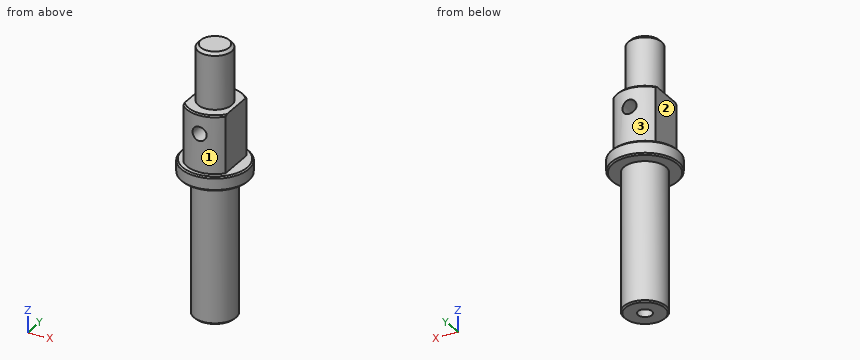
```python
from build123d import *

# Parameters (mm, degrees)
SKETCH_1_R             = 7.5
EXTRUDE_1_DEPTH        = 49.5
SKETCH_2_R             = 12
EXTRUDE_2_DEPTH        = 5
SKETCH_3_R             = 10
EXTRUDE_3_DEPTH        = 20.5
SKETCH_4_R             = 6
EXTRUDE_4_DEPTH        = 20
HOLE_WIZARD_M6_1_D     = 5
HOLE_WIZARD_M6_1_DEPTH = 15
HOLE_WIZARD_M6_1_TIP   = 1.502151548
CHAMFER_1_SIZE         = 0.5
CHAMFER_2_SIZE         = 1
CHAMFER_3_SIZE         = 0.5
SKETCH_7_W             = 26.460285879
SKETCH_7_H             = 26.47281766
SKETCH_7_W_2           = 19.498728734
SKETCH_7_H_2           = 28.747669346
CUT_EXTRUDE_1_DEPTH    = 52
HOLE_WIZARD_M6_2_D     = 5


with BuildPart() as part:
    # 草图1 → 凸台-拉伸1 (new body)
    with BuildSketch(Plane.XY):
        Circle(SKETCH_1_R)
    extrude(amount=EXTRUDE_1_DEPTH)

    # 草图2 → 凸台-拉伸2 (add)
    with BuildSketch(Plane.XY.offset(49.5)):
        Circle(SKETCH_2_R)
    extrude(amount=EXTRUDE_2_DEPTH)

    # 草图3 → 凸台-拉伸3 (add)
    with BuildSketch(Plane.XY.offset(54.5)):
        Circle(SKETCH_3_R)
    extrude(amount=EXTRUDE_3_DEPTH)

    # 草图4 → 凸台-拉伸4 (add)
    with BuildSketch(Plane.XY.offset(75)):
        Circle(SKETCH_4_R)
    extrude(amount=EXTRUDE_4_DEPTH)

    # M6 螺纹孔1
    with Locations(Plane(origin=(0, 0, 0), x_dir=(-1, 0, 0), z_dir=(0, 0, -1))):
        with Locations((0, 0)):
            Hole(HOLE_WIZARD_M6_1_D / 2, depth=HOLE_WIZARD_M6_1_DEPTH)
            with Locations((0, 0, -(HOLE_WIZARD_M6_1_DEPTH + HOLE_WIZARD_M6_1_TIP / 2))):  # 118° drill point
                Cone(0, HOLE_WIZARD_M6_1_D / 2, HOLE_WIZARD_M6_1_TIP, mode=Mode.SUBTRACT)

    # 倒角1
    chamfer_1_edges = [part.edges().sort_by_distance(p)[0] for p in [
        (-7.5, 0, 0),
        (-12, 0, 49.5),
        (-12, 0, 54.5),
    ]]
    chamfer(chamfer_1_edges, length=CHAMFER_1_SIZE)

    # 倒角2
    chamfer_2_edges = [part.edges().sort_by_distance(p)[0] for p in [
        (-6, 0, 95),
    ]]
    chamfer(chamfer_2_edges, length=CHAMFER_2_SIZE)

    # 倒角3
    chamfer_3_edges = [part.edges().sort_by_distance(p)[0] for p in [
        (-10, 0, 75),
    ]]
    chamfer(chamfer_3_edges, length=CHAMFER_3_SIZE)

    # 草图7 → 切除-拉伸1 (cut, symmetric)
    with BuildSketch(Plane(origin=(0, 0, 0), x_dir=(1, 0, 0), z_dir=(0, 1, 0))):
        with Locations((-20.73014294, -67.73640883)):
            Rectangle(SKETCH_7_W, SKETCH_7_H)
        with Locations((17.249364367, -68.873834673)):
            Rectangle(SKETCH_7_W_2, SKETCH_7_H_2)
    extrude(amount=CUT_EXTRUDE_1_DEPTH, both=True, mode=Mode.SUBTRACT)

    # M6 螺纹孔2 (through all)
    with Locations(Plane(origin=(0, 10, 0), x_dir=(1, 0, 0), z_dir=(0, 1, 0))):
        with Locations((0, -68)):
            Hole(HOLE_WIZARD_M6_2_D / 2)


solid = part.part
```
Source: CAD feature listing. Evaluate the final solid. Frame: model axes, mm. Face numbers are marked on the shaded views. A direction names the side the tool comes from. Coordinates: 2 decimals unless noted, no trailing zeros. Loops run counter-clockwise (first coordinate to the right, second up) from the corner with the lowest first, then second, coordinate; pieces in that order, holes last. Notation, with made-up numbers: (-29.5, 43.5) -> (-19.5, 43.5) arc R21 cw to (-19.5, 82.5) -> close; hole circle Ø3 at (61.25, 40). An arc over 180 degrees is marked (long way). One line per item, written item: value. Start each with the question number.
Q1. Line query: line 1 along Z through (x, y) = (0, -2.75); line 2 along Y through (x, z) = (0, 4.5). Output: solid intervals per line, ascending.
Q2. Contact query for flat-ended pins moving along their axis: P1, Ø8, axis at x = 2.5, z = 30.5, coming from the -Y side; P2, Ø12, axis at x = 4, z = 23, coming from the +Y side; P3, Ø6, axis at y = -3.5, z = 72.5, coming from the -X side; P4, Ø3, axis at y = 9.5, z = 31.5, coming from the -X side. Output: stop coordinate, or through.
Q3. Set-up query: the marked faces 1, 2 and 3. Return all of +Z, -Z, +X, -X, +Y, -Y with unobstructed straight access to the full face (end or side cutting, diameter ignored); none if empty.
Q4. Section query A-A, the plane z = 68. Return the cut outline in (x, y), and give its area (3 significant figures).
Q5. Section query B-B, the plane z = 51. Return the cut outline in (x, y), and give its area (3 significant figures).
Q6. Section query C-C, the plane z = 81.5. Return the cut outline in (x, y).
Results:
1. line 1: 0 to 65.5, 70.5 to 95
1. line 2: -7.5 to -2.5, 2.5 to 7.5
2. P1: y = -7.5
2. P2: y = 7.5
2. P3: x = -7.5
2. P4: through
3. face 1: +Z, -Y
3. face 2: +Z, -X, +Y, -Y
3. face 3: +Z, +Y
4. outline: (-7.5, -6.61) arc R10 ccw to (-2.5, -9.68) -> (-2.5, 9.68) arc R10 ccw to (-7.5, 6.61) -> close; (2.5, -9.68) arc R10 ccw to (7.5, -6.61) -> (7.5, 6.61) arc R10 ccw to (2.5, 9.68) -> close
4. area: 170 mm^2
5. outline: circle Ø24 at (0, 0)
5. area: 452 mm^2
6. outline: circle Ø12 at (0, 0)
